The model under review builds one solid part; all positions refer to its coordinate system, in mm. A direction names the side the tool comes from. Round coordinates to 2 decimals unless told otherwise and drop trailing zeros. Write each loop counter-clockwise with the first axis right and the second up, starting at its lowest first coordinate (ties: lowest second). Pieces come first, ordered by that corner, then holes. Notation, with made-up numbers: (48.25, -15.75) -> (80.25, -15.75) arc R18 cw to (80.25, -6.75) -> close; hole circle Ø2 at (11, 3). An arc over 180 degrees is marked (long way). Return JSON: item names as keys, results as strings. Group by question number.
1. Take a section at B-B, the plane x = 69. Write out the cut boundary in (y, z), then the cut area to 3 significant figures.
2. For line 1 along Z through (x, y) = (32.5, 5.5); line 2 along X through (y, z) = (-5.25, 7.25); line 3 along Y through (x, z) = (4, -1.5), list the stretches that pass through material, from the lowest coordinate up. Write a range as from..to.
3. Tool access review of faces 1 (the conical face through (7.97, 5.18, 8.92)), 2 (the cylindrical face through (42.78, 3.86, -5.04)): name each direction out of +Z, -Z, +X, -X, +Y, -Y from which nothing blocks a thin tool from reaching the whole face with its end or side.
4. Take a section at A-A, the plane y = 0. Write out the cut boundary in (x, z) (3 decimals), then the cut area to 3 significant figures.
5. Clearance check with flat-ended pins moving along their axes: P1, Ø5, axis at y = 5, z = -3.5, coming from the -X side; P2, Ø6, axis at x = 41, z = -1, coming from the -Y side; P3, Ø10, axis at x = 33, y = -2.5, coming from the +Z side; P4, Ø5, axis at x = 15.5, z = -7, coming from the +Y side. State where each tip first meets the part, or that it passes through.
from build123d import *

# Parameters (mm, degrees)
BASE_EXTRUDE_DEPTH = 8.73125
SKETCH4_W          = 0.6
SKETCH4_H          = 11.998522628
CHAMFER_2_SIZE     = 1.4
FILLET_2_R         = 0.6


with BuildPart() as part:
    # Sketch1 → Base-Extrude (new body)
    with BuildSketch(Plane(origin=(0, 0, 0), x_dir=(0, 0, -1), z_dir=(1, 0, 0))):
        Polygon((9.525, 5.499261314), (9.525, -5.499261314), (0, -10.998522628), (-9.525, -5.499261314), (-9.525, 5.499261314), (0, 10.998522628), align=None)
    extrude(amount=BASE_EXTRUDE_DEPTH)

    # Sketch2 → Boss-Revolve1 (revolve)
    with BuildSketch(Plane.XY, mode=Mode.PRIVATE) as boss_revolve1_sk:
        Polygon((0, 0), (78.58125, 0), (78.58125, 5.55625), (78.58125, 6.35), (27.8072, 6.35), (0, 6.35), align=None)
    revolve(boss_revolve1_sk.sketch.rotate(Axis((0, 0, 0), (1, 0, 0)), 90), axis=Axis((0, 0, 0), (1, 0, 0)))

    # Sketch3 → Cut-Revolve1 (revolve, cut)
    with BuildSketch(Plane.XY, mode=Mode.PRIVATE) as cut_revolve1_sk:
        Polygon((0, 9), (4.040598923, 15.998522628), (4.040598923, 20.998522628), (-10, 20.998522628), (-10, 9), align=None)
    revolve(cut_revolve1_sk.sketch.rotate(Axis((0, 0, 0), (1, 0, 0)), 300.000000006), axis=Axis((0, 0, 0), (1, 0, 0)), mode=Mode.SUBTRACT)

    # Sketch5 → Cut-Revolve2 (revolve, cut)
    with BuildSketch(Plane.XY, mode=Mode.PRIVATE) as cut_revolve2_sk:
        Polygon((8.73125, 9), (4.690651077, 15.998522628), (4.690651077, 20.998522628), (14.690651077, 20.998522628), (14.690651077, 9), align=None)
    revolve(cut_revolve2_sk.sketch.rotate(Axis((0, 0, 0), (1, 0, 0)), 90), axis=Axis((0, 0, 0), (1, 0, 0)), mode=Mode.SUBTRACT)

    # Sketch4 → Cut-Revolve3 (revolve, cut)
    with BuildSketch(Plane.XY, mode=Mode.PRIVATE) as cut_revolve3_sk:
        with Locations((8.43125, 14.999261314)):
            Rectangle(SKETCH4_W, SKETCH4_H)
    revolve(cut_revolve3_sk.sketch.rotate(Axis((0, 0, 0), (1, 0, 0)), 90), axis=Axis((0, 0, 0), (1, 0, 0)), mode=Mode.SUBTRACT)

    # Chamfer 2
    chamfer_2_edges = [part.edges().sort_by_distance(p)[0] for p in [
        (78.58125, 0, -6.35),
    ]]
    chamfer(chamfer_2_edges, length=CHAMFER_2_SIZE)

    # Fillet 2
    fillet_2_edges = [part.edges().sort_by_distance(p)[0] for p in [
        (8.73125, 0, -6.35),
    ]]
    fillet(fillet_2_edges, radius=FILLET_2_R)


solid = part.part
Output:
{
 "1": {"outline": "circle Ø12.7 at (0, 0)", "area": "127 mm^2"},
 "2": {"line 1": "z = -3.17..3.17", "line 2": "x = 0..8.73", "line 3": "y = -10.13..10.13"},
 "3": {"face 1": "+Z, +X, +Y", "face 2": "+X"},
 "4": {"outline": "(0, -9) -> (0.303, -9.525) -> (8.131, -9.525) -> (8.131, -9) -> (8.731, -9) -> (8.731, -6.95) arc R0.6 cw to (9.331, -6.35) -> (77.181, -6.35) -> (78.581, -4.95) -> (78.581, 4.95) -> (77.181, 6.35) -> (9.331, 6.35) arc R0.6 cw to (8.731, 6.95) -> (8.731, 9) -> (8.131, 9) -> (8.131, 9.525) -> (0.303, 9.525) -> (0, 9) -> close", "area": "1,050 mm^2"},
 "5": {"P1": "stops at x = 0", "P2": "stops at y = -6.35", "P3": "stops at z = 6.35", "P4": "stops at y = 4.48"}
}
